```python
from build123d import *

# Parameters (mm, degrees)
SKETCH_1_W                = 23
SKETCH_1_H                = 22
EXTRUDE_1_DEPTH           = 445
HOLE_WIZARD_1_D           = 6.6
HOLE_WIZARD_1_CBORE_D     = 11
HOLE_WIZARD_1_CBORE_DEPTH = 6.8
PATTERN_LINEAR_1_COUNT    = 8
PATTERN_LINEAR_1_PITCH    = 60


with BuildPart() as part:
    # 草图1 → 凸台-拉伸1 (new body)
    with BuildSketch(Plane.XY):
        with Locations((0, 11)):
            Rectangle(SKETCH_1_W, SKETCH_1_H)
    extrude(amount=EXTRUDE_1_DEPTH)

    # 打孔尺寸(%根据)内六角圆柱头螺钉的类型1 (through all)
    with Locations(Plane(origin=(0, 22, 0), x_dir=(1, 0, 0), z_dir=(0, 1, 0))):
        with Locations((0, -402.5)):
            hole_wizard_1 = CounterBoreHole(HOLE_WIZARD_1_D / 2, HOLE_WIZARD_1_CBORE_D / 2, HOLE_WIZARD_1_CBORE_DEPTH)

    # 阵列(线性)1: 打孔尺寸(%根据)内六角圆柱头螺钉的类型1 ×8
    with Locations(*[(0, 0, -i * PATTERN_LINEAR_1_PITCH) for i in range(1, PATTERN_LINEAR_1_COUNT)]):
        add(hole_wizard_1, mode=Mode.SUBTRACT)


solid = part.part
```
The model under review builds one solid part; all positions refer to its coordinate system, in mm. A direction names the side the tool comes from. Coordinates: 2 decimals unless noted, no trailing zeros. Write each loop counter-clockwise with the first axis right and the second up, starting at its lowest first coordinate (ties: lowest second). Pieces come first, ordered by that corner, then holes. Notation, with made-up numbers: (4.5, 41) - (29.5, 41) arc R24 ccw to (29.5, 63) - close; hole circle Ø8 at (-34, -28.5). An arc over 180 degrees is marked (long way). Answer in a Markdown table with one row per item. Add a question column.
Q1. Consider section A-A on y = 4. Give the boundary of the cut face in (x, z).
Q2. To check wall thickness, follow line 1 along X through (y, z) = (18, 402.5); line 2 along X through (y, z) = (9, 342.5). State the ranges of each line that lie inside material, in increasing order. Write a range as from..to.
Q3. For faces 1 (the face through (-5, 22, 219)), 2 (the face through (4, 15.2, 102)), list the 3-axis set-ups (+Z, -Z, +X, -X, +Y, -Y) from which the entire face can be reached by the end or side of a thin tool; tool diameter is ignored.
Q4. Clearance check with flat-ended pins moving along their axes: pin 1 (10 mm diameter, centred on x = 0, z = 402.5, fed in from +Y); pin 2 (5.5 mm diameter, centred on x = 0, z = 42.5, fed in from +Y). State where each tip first meets the part, or that it passes through.
Answers below:
| question | item | result |
|---|---|---|
| 1 | outline | (-11.5, 0) - (11.5, 0) - (11.5, 445) - (-11.5, 445) - close; hole circle Ø6.6 at (0, 42.5); hole circle Ø6.6 at (0, 102.5); hole circle Ø6.6 at (0, 162.5); hole circle Ø6.6 at (0, 222.5); hole circle Ø6.6 at (0, 282.5); hole circle Ø6.6 at (0, 342.5); hole circle Ø6.6 at (0, 402.5) |
| 2 | line 1 | -11.5..-5.5, 5.5..11.5 |
| 2 | line 2 | -11.5..-3.3, 3.3..11.5 |
| 3 | face 1 | +Z, -Z, +X, -X, +Y |
| 3 | face 2 | +Y |
| 4 | pin 1 | y = 15.2 |
| 4 | pin 2 | through |
